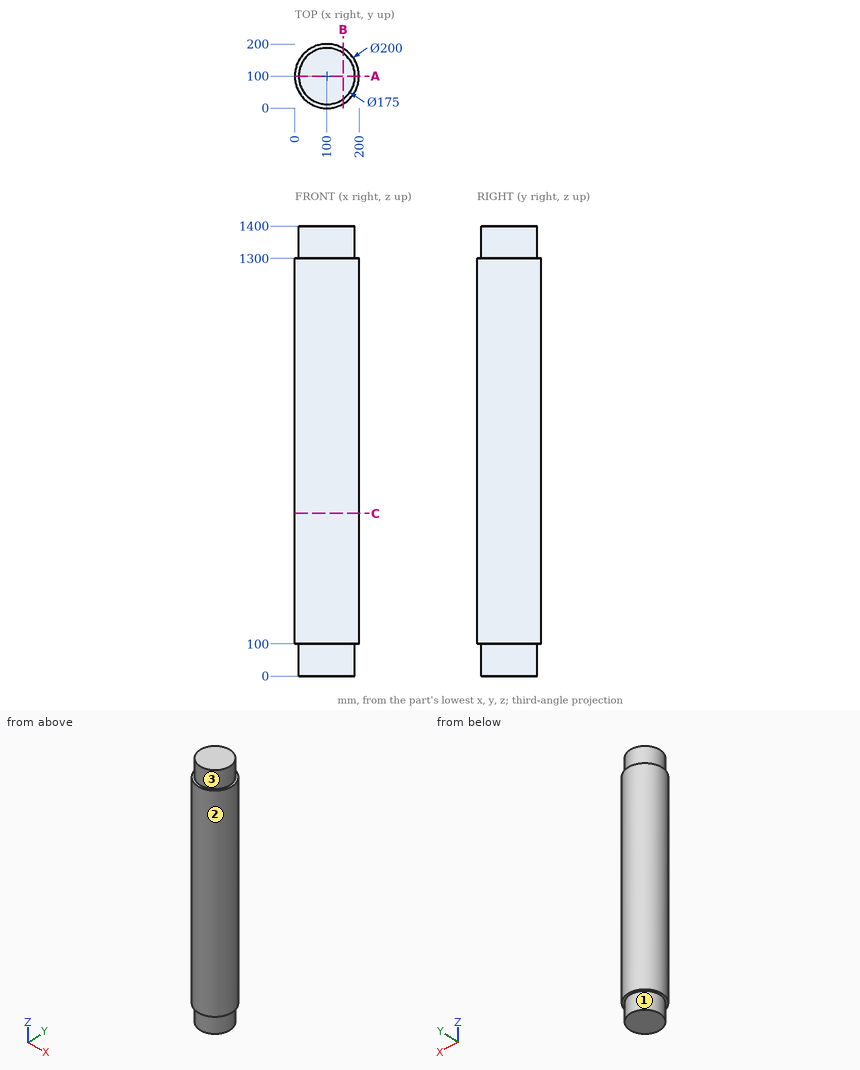
Verification items for this drawing (mm, ordinates from the low corner). A direction names the side the tool comes from. Round coordinates to 2 decimals unless told otherwise and drop trailing zeros. Loops run counter-clockwise (first coordinate to the right, second up) from the corner with the lowest first, then second, coordinate; pieces in that order, holes last. Notation, with made-up numbers: M 34,88 L 81,88 A15 ccw 81,100 Z; hole C -17.75,53 d5. An arc over 180 degrees is marked long. Answer as a JSON object with one key per item and string values.
1. Scan lines: line 1 (X direction, y = 98, z = 923.5); line 2 (X direction, y = 106.5, z = 200.5); line 3 (Z direction, x = 83, y = 190). Record each from-to range of solid material in increasing order.
Reply:
{"line 1": "x = 0.02 to 199.98", "line 2": "x = 0.21 to 199.79", "line 3": "z = 100 to 1300"}
2. Access from +Z, -Z, +X, -X, +Y, -Y to the whole of each face (thin tool, end or side, straight path). Record for the marked faces 1, 2 and 3.
Reply:
{"face 1": "-Z", "face 2": "+Z, -Z", "face 3": "+Z"}
3. Section check A-A (y = 100). Record the boundary of the cut face in (x, z), plus the area to 3 significant figures.
Reply:
{"outline": "M 0,100 L 12.5,100 L 12.5,0 L 187.5,0 L 187.5,100 L 200,100 L 200,1300 L 187.5,1300 L 187.5,1400 L 12.5,1400 L 12.5,1300 L 0,1300 Z", "area": "275,000 mm²"}
4. Section check C-C (z = 506). Record the boundary of the cut face in (x, y), plus the area to 3 significant figures.
Reply:
{"outline": "C 100,100 d200", "area": "31,400 mm²"}
5. Section check B-B (x = 150.5). Record the boundary of the cut face in (y, z).
Reply:
{"outline": "M 13.69,100 L 28.54,100 L 28.54,0 L 171.46,0 L 171.46,100 L 186.31,100 L 186.31,1300 L 171.46,1300 L 171.46,1400 L 28.54,1400 L 28.54,1300 L 13.69,1300 Z"}
6. Gauge pin test, flat ends, axial feed: P1, Ø8, axis at y = 167, z = 932.5, coming from the -X side; P2, Ø3, axis at y = 20.5, z = 187, coming from the -X side; P3, Ø1.5, axis at x = 72, z = 1031.5, coming from the +Y side. Record the tip position at first contact, or that the pin passes through.
Reply:
{"P1": "stops at x = 22.34", "P2": "stops at x = 37.42", "P3": "stops at y = 196.22"}
